Could you check a few things on this drawing? It's one solid part, dimensions in mm from its lowest x, y, z. Coordinates: 2 decimals unless noted, no trailing zeros. Order: outer loops, then holes, each group sorted by start corner. A loop starts at its lowest first (then second) coordinate and runs counter-clockwise, first axis right, second up.
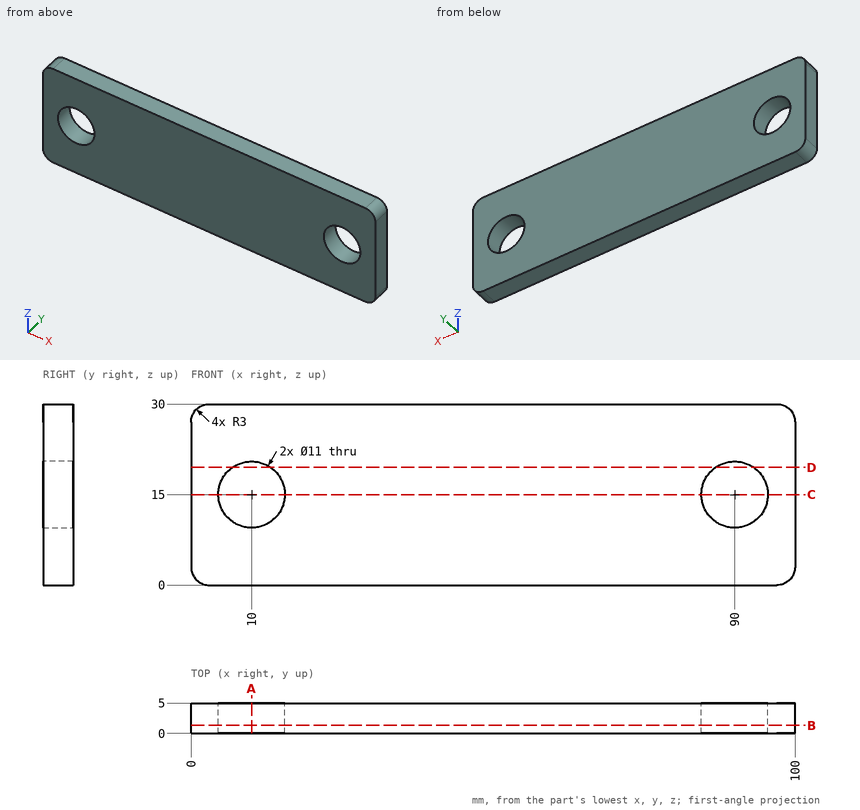
1. Imagine slicing it at C-C on z = 15. Please give me the cut outline in (x, y), then the cut area to 3 significant figures.
Completed:
outline: (0, 0) - (4.5, 0) - (4.5, 5) - (0, 5) - close; (15.5, 0) - (84.5, 0) - (84.5, 5) - (15.5, 5) - close; (95.5, 0) - (100, 0) - (100, 5) - (95.5, 5) - close
area: 390 mm2
2. I'm going to push a flat-ended pin straight in: pin 1 (1.5 mm diameter, centred on x = 44.5, z = 4.5, fed in from -Y). Where does the tip first touch, or does it pass through?
Completed:
pin 1: stops at y = 0
3. Imagine slicing it at B-B on y = 1.3. Please give me the cut outline in (x, z).
Completed:
outline: (0, 3) arc R3 ccw to (3, 0) - (97, 0) arc R3 ccw to (100, 3) - (100, 27) arc R3 ccw to (97, 30) - (3, 30) arc R3 ccw to (0, 27) - close; hole circle Ø11 at (10, 15); hole circle Ø11 at (90, 15)
4. Imagine slicing it at D-D on z = 19.5. Please give me the cut outline in (x, y), then the cut area to 3 significant figures.
Completed:
outline: (0, 0) - (6.84, 0) - (6.84, 5) - (0, 5) - close; (13.16, 0) - (86.84, 0) - (86.84, 5) - (13.16, 5) - close; (93.16, 0) - (100, 0) - (100, 5) - (93.16, 5) - close
area: 437 mm2
5. Please list where these lines run through material, in increasing order: probe 1 along X at (y, z) = (1.8, 15); probe 2 along Z at (x, y) = (12, 2.75); probe 3 along Z at (x, y) = (15, 4.75).
Completed:
probe 1: x = 0 to 4.5, 15.5 to 84.5, 95.5 to 100
probe 2: z = 0 to 9.88, 20.12 to 30
probe 3: z = 0 to 12.71, 17.29 to 30
6. Imagine slicing it at A-A on x = 10. Please give me the cut outline in (y, z).
Completed:
outline: (0, 0) - (5, 0) - (5, 9.5) - (0, 9.5) - close; (0, 20.5) - (5, 20.5) - (5, 30) - (0, 30) - close
